Read the model definition and answer for the solid it produces. Units are mm, in the model's axes. Face numbers are marked on the shaded views. A direction names the side the tool comes from. Coordinates: 2 decimals unless noted, no trailing zeros. Order: outer loops, then holes, each group sorted by start corner. A loop starts at its lowest first (then second) coordinate and runs counter-clockwise, first axis right, second up. Notation, with made-up numbers: M -20,-16.75 L 26,-16.75 A29 cw 26,18.25 Z; hole C 66,-12 d5. An arc over 180 degrees is marked long. One line per question, with ' | ' between items. Start each with the question number.
1) Given P1, Ø4, axis at x = 11.31, y = 11.31, coming from the -Z side; P2, Ø10, axis at y = 2.5, z = 12.5, coming from the +X side; P3, Ø3, axis at x = 9, y = 9, coming from the -Z side, each flat-ended and moving along its own axis, determine where each tip first touches the part or whether it passes through.
2) Consider probe 1 along Y at (x, z) = (0, 3.75); probe 2 along X at (y, z) = (7.5, 10); probe 3 along Z at (x, y) = (11.5, -13). Determine where each line is inside the solid, lowest interval first.
3) Find section A-A, the plane x = 0. Write down the section's boundary in (y, z) (3 decimals).
4) Find section D-D, the plane z = 9.5. Write down the section's boundary in (x, y).
5) Find section C-C, the plane z = 12.5. Count the separate pieces of the cut face and the enclosed holes in it, plus the area to 3 significant figures.
6) The mould has two halves that part along X. Classify the marked faces 4, 5 and 6: +X half, -X half, draft (parallel to the pull), parting line (faces both ways), or undercut.
7) A tool of negligible diameter and unlimited length cuts with its end or side. For the marked faces 1, 2 and 3, from which of +Z, -Z, +X, -X, +Y, -Y can it reach the whole face along a straight path? Write none if from no direction.
from build123d import *
from build123d.topology import SkipClean

# Parameters (mm, degrees)
SKETCH_1_R          = 11
SKETCH_1_R_2        = 9
EXTRUDE_1_DEPTH     = 6.8
SKETCH_2_R          = 12.5
SKETCH_2_R_2        = 9
EXTRUDE_2_DEPTH     = 8
SKETCH_4_R          = 12.5
SKETCH_4_R_2        = 9
EXTRUDE_3_DEPTH     = 5
CUT_EXTRUDE_START   = -5
SKETCH_8_R          = 12.5
SKETCH_8_R_2        = 9
CUT_EXTRUDE_1_DEPTH = 5
EXTRUDE_START       = -3.5
EXTRUDE_4_DEPTH     = 3.5
HOLE_WIZARD_M3_1_D  = 2.5
FILLET_1_R          = 3
EXTRUDE_START_2     = 1.2
SKETCH_13_R         = 10.075
SKETCH_13_R_2       = 9
EXTRUDE_5_DEPTH     = 1.2
EXTRUDE_START_3     = 2
SKETCH_14_R         = 11
SKETCH_14_R_2       = 9
EXTRUDE_6_DEPTH     = 2
CHAMFER_2_SIZE      = 0.5


with BuildPart() as part:
    # 草图1 → 凸台-拉伸1 (new body)
    with BuildSketch(Plane.XY):
        Circle(SKETCH_1_R)
        Circle(SKETCH_1_R_2, mode=Mode.SUBTRACT)
    extrude(amount=EXTRUDE_1_DEPTH)

    # 草图2 → 凸台-拉伸2 (add)
    with BuildSketch(Plane.XY.offset(6.8)):
        Circle(SKETCH_2_R)
        Circle(SKETCH_2_R_2, mode=Mode.SUBTRACT)
    extrude(amount=EXTRUDE_2_DEPTH)

    # 草图4 → 凸台-拉伸3 (add)
    with BuildSketch(Plane.XY.offset(14.8)):
        Circle(SKETCH_4_R)
        Circle(SKETCH_4_R_2, mode=Mode.SUBTRACT)
    extrude(amount=EXTRUDE_3_DEPTH)

    # 草图8 → 切除-拉伸1 (cut)
    with BuildSketch(Plane.XY.offset(19.8).offset(CUT_EXTRUDE_START)):
        Circle(SKETCH_8_R)
        Circle(SKETCH_8_R_2, mode=Mode.SUBTRACT)
    extrude(amount=CUT_EXTRUDE_1_DEPTH, mode=Mode.SUBTRACT)

    # 草图9 → 凸台-拉伸4 (add)
    with BuildSketch(Plane.XY.offset(14.8).offset(EXTRUDE_START)):
        with BuildLine():
            Line((10.966125931, 15.208766619), (6.459180807, 10.701821494))
            ThreePointArc((6.459180807, 10.701821494), (8.838834765, 8.838834765), (10.701821494, 6.459180807))
            Line((10.701821494, 6.459180807), (15.208766619, 10.966125931))
            ThreePointArc((15.208766619, 10.966125931), (13.258252147, 13.258252147), (10.966125931, 15.208766619))
        make_face()
        with BuildLine():
            Line((15.208766619, -10.966125931), (10.701821494, -6.459180807))
            ThreePointArc((10.701821494, -6.459180807), (8.838834765, -8.838834765), (6.459180807, -10.701821494))
            Line((6.459180807, -10.701821494), (10.966125931, -15.208766619))
            ThreePointArc((10.966125931, -15.208766619), (13.258252147, -13.258252147), (15.208766619, -10.966125931))
        make_face()
        with BuildLine():
            Line((-10.966125931, -15.208766619), (-6.459180807, -10.701821494))
            ThreePointArc((-6.459180807, -10.701821494), (-8.838834765, -8.838834765), (-10.701821494, -6.459180807))
            Line((-10.701821494, -6.459180807), (-15.208766619, -10.966125931))
            ThreePointArc((-15.208766619, -10.966125931), (-13.258252147, -13.258252147), (-10.966125931, -15.208766619))
        make_face()
        with BuildLine():
            Line((-15.208766619, 10.966125931), (-10.701821494, 6.459180807))
            ThreePointArc((-10.701821494, 6.459180807), (-8.838834765, 8.838834765), (-6.459180807, 10.701821494))
            Line((-6.459180807, 10.701821494), (-10.966125931, 15.208766619))
            ThreePointArc((-10.966125931, 15.208766619), (-13.258252147, 13.258252147), (-15.208766619, 10.966125931))
        make_face()
    extrude(amount=EXTRUDE_4_DEPTH)

    # M3 螺纹孔1 (through all)
    with Locations(Plane.XY.offset(14.8)):
        with Locations((-11.313708499, 11.313708499), (11.313708499, 11.313708499), (11.313708499, -11.313708499), (-11.313708499, -11.313708499)):
            Hole(HOLE_WIZARD_M3_1_D / 2)

    # 圆角1
    fillet_1_edges = [part.edges().sort_by_distance(p)[0] for p in [
        (10.701821494, 6.459180807, 13.05),
        (6.459180807, 10.701821494, 13.05),
        (6.459180807, -10.701821494, 13.05),
        (10.701821494, -6.459180807, 13.05),
        (-10.701821494, -6.459180807, 13.05),
        (-6.459180807, -10.701821494, 13.05),
        (-6.459180807, 10.701821494, 13.05),
        (-10.701821494, 6.459180807, 13.05),
    ]]
    fillet(fillet_1_edges, radius=FILLET_1_R)

    # 草图13 → 凸台-拉伸5 (add)
    with SkipClean():  # the faces are left unmerged after this step: merging them gives an invalid solid
        with BuildSketch(Plane(origin=(0, 0, 0), x_dir=(-1, 0, 0), z_dir=(0, 0, -1)).offset(EXTRUDE_START_2)):
            with Locations(Location((0, 0, 0), (0, 0, 180))):
                Circle(SKETCH_13_R)
            Circle(SKETCH_13_R_2, mode=Mode.SUBTRACT)
        extrude(amount=-EXTRUDE_5_DEPTH)

    # 草图14 → 凸台-拉伸6 (add)
    with SkipClean():  # the faces are left unmerged after this step: merging them gives an invalid solid
        with BuildSketch(Plane(origin=(0, 0, -1.2), x_dir=(-1, 0, 0), z_dir=(0, 0, -1)).offset(EXTRUDE_START_3)):
            with Locations(Location((0, 0, 0), (0, 0, 180))):
                Circle(SKETCH_14_R)
            Circle(SKETCH_14_R_2, mode=Mode.SUBTRACT)
        extrude(amount=-EXTRUDE_6_DEPTH)

    # 倒角2
    chamfer_2_edges = [part.edges().sort_by_distance(p)[0] for p in [
        (-11, 0, -3.2),
    ]]
    chamfer(chamfer_2_edges, length=CHAMFER_2_SIZE)


solid = part.part
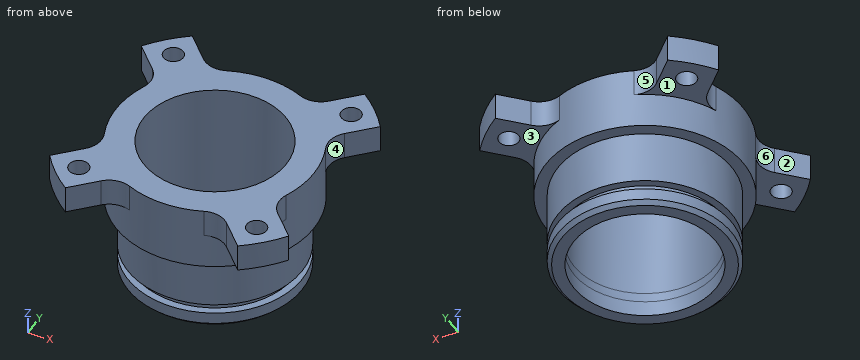
Report:
1) P1: stops at z = 11.3 | P2: stops at x = 12.5 | P3: stops at z = 6.8
2) probe 1: y = -11 to -9, 9 to 11 | probe 2: x = -10 to -4.97, 4.97 to 10 | probe 3: z = 11.3 to 14.8
3) outline: M -12.5,6.8 L -11,6.8 L -11,0 L -10.075,0 L -10.075,-1.2 L -11,-1.2 L -11,-2.7 L -10.5,-3.2 L -9,-3.2 L -9,14.8 L -12.5,14.8 Z; M 9,-3.2 L 10.5,-3.2 L 11,-2.7 L 11,-1.2 L 10.075,-1.2 L 10.075,0 L 11,0 L 11,6.8 L 12.5,6.8 L 12.5,14.8 L 9,14.8 Z
4) outline: C 0,0 d25; hole C 0,0 d18
5) separate pieces: 1 | enclosed holes: 5 | area: 374 mm^2
6) face 4: +X half | face 5: undercut | face 6: -X half
7) face 1: -Z, -X, +Y | face 2: +Z, -Z, -X | face 3: -Z, +X, +Y
